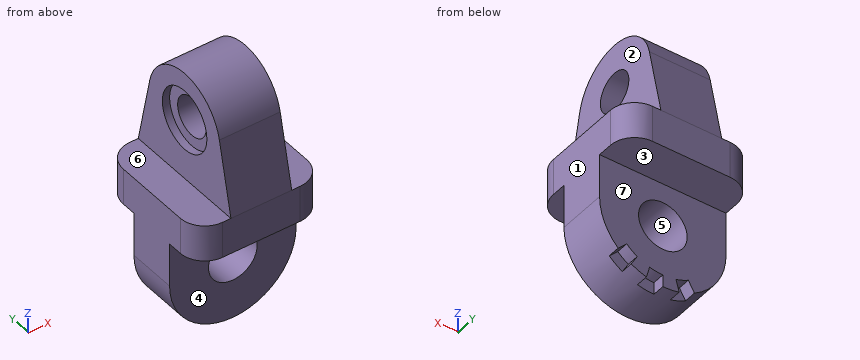
```python
from build123d import *

# Parameters (mm, degrees)
ROUNDED_BASE_BLOCK_DEPTH   = 15
UPPER_BLOCK_DEPTH          = 52
UPPER_BLOCK_NOTCH_A_DEPTH  = 13.5
UPPER_START                = -13.5
UPPER_BLOCK_NOTCH_B_DEPTH  = 13.5
CROSS_BLOCK_DEPTH          = 52
CROSS_BLOCK_NOTCH_A_DEPTH  = 16
CROSS_START                = -16
CROSS_BLOCK_NOTCH_B_DEPTH  = 16
BORE_NOTCH_TEETH_CUT_DEPTH = 5
CROSS_BORE_10_SKETCH_R     = 10
CROSS_BORE_10_DEPTH        = 50
COUNTERBORE_25_SKETCH_R    = 12.5
COUNTERBORE_25_X3_DEPTH    = 3
MAIN_BORE_16_SKETCH_R      = 8
MAIN_BORE_16_DEPTH         = 50


with BuildPart() as part:
    # Base Block Profile Sketch → Rounded Base Block (new body)
    with BuildSketch(Plane.XY):
        with BuildLine():
            Line((-16, 0), (16, 0))
            ThreePointArc((16, 0), (23.071067812, 2.928932188), (26, 10))
            Line((26, 10), (26, 42))
            ThreePointArc((26, 42), (23.071067812, 49.071067812), (16, 52))
            Line((16, 52), (-16, 52))
            ThreePointArc((-16, 52), (-23.071067812, 49.071067812), (-26, 42))
            Line((-26, 42), (-26, 10))
            ThreePointArc((-26, 10), (-23.071067812, 2.928932188), (-16, 0))
        make_face()
    extrude(amount=ROUNDED_BASE_BLOCK_DEPTH)

    # Upper Block Profile Sketch → Upper Block (add)
    with BuildSketch(Plane.ZY.offset(26)):
        with BuildLine():
            Line((15, 52), (15, 0))
            Line((15, 0), (44.311040938, 6.470152944))
            ThreePointArc((44.311040938, 6.470152944), (60, 26), (44.311040938, 45.529847056))
            Line((44.311040938, 45.529847056), (15, 52))
        make_face()
    extrude(amount=-UPPER_BLOCK_DEPTH)

    # Upper Block Notch A Sketch → Upper Block Notch A (cut)
    with BuildSketch(Plane.ZY.offset(26)):
        with BuildLine():
            Line((15, 52), (44.311040938, 45.529847056))
            ThreePointArc((44.311040938, 45.529847056), (60, 26), (44.311040938, 6.470152944))
            Line((44.311040938, 6.470152944), (15, 0))
            Line((15, 0), (15, 52))
        make_face()
    extrude(amount=-UPPER_BLOCK_NOTCH_A_DEPTH, mode=Mode.SUBTRACT)

    # Upper Block Notch B Sketch → Upper Block Notch B (cut)
    with BuildSketch(Plane(origin=(26, 0, 0), x_dir=(0, 0, -1), z_dir=(1, 0, 0)).offset(UPPER_START)):
        with BuildLine():
            Line((-15, 52), (-15, 0))
            Line((-15, 0), (-44.311040938, 6.470152944))
            ThreePointArc((-44.311040938, 6.470152944), (-60, 26), (-44.311040938, 45.529847056))
            Line((-44.311040938, 45.529847056), (-15, 52))
        make_face()
    extrude(amount=UPPER_BLOCK_NOTCH_B_DEPTH, mode=Mode.SUBTRACT)

    # Cross Block Profile Sketch → Cross Block (add)
    with BuildSketch(Plane(origin=(0, 52, 0), x_dir=(1, 0, 0), z_dir=(0, 1, 0))):
        with BuildLine():
            Line((-26, 0), (-26, 18))
            ThreePointArc((-26, 18), (0, 44), (26, 18))
            Line((26, 18), (26, 0))
            Line((26, 0), (-26, 0))
        make_face()
    extrude(amount=-CROSS_BLOCK_DEPTH)

    # Cross Block Notch A Sketch → Cross Block Notch A (cut)
    with BuildSketch(Plane(origin=(0, 52, 0), x_dir=(1, 0, 0), z_dir=(0, 1, 0))):
        with BuildLine():
            Line((-26, 0), (26, 0))
            Line((26, 0), (26, 18))
            ThreePointArc((26, 18), (0, 44), (-26, 18))
            Line((-26, 18), (-26, 0))
        make_face()
    extrude(amount=-CROSS_BLOCK_NOTCH_A_DEPTH, mode=Mode.SUBTRACT)

    # Cross Block Notch B Sketch → Cross Block Notch B (cut)
    with BuildSketch(Plane.XZ.offset(CROSS_START)):
        with BuildLine():
            Line((-26, 0), (26, 0))
            Line((26, 0), (26, -18))
            ThreePointArc((26, -18), (0, -44), (-26, -18))
            Line((-26, -18), (-26, 0))
        make_face()
    extrude(amount=CROSS_BLOCK_NOTCH_B_DEPTH, mode=Mode.SUBTRACT)

    # Bore Notch Teeth Sketch → Bore Notch Teeth Cut (cut)
    with BuildSketch(Plane(origin=(0, 36, 0), x_dir=(1, 0, 0), z_dir=(0, 1, 0))):
        with BuildLine():
            Line((-5.435199947, 38.284442352), (-6.729295173, 43.114071484))
            ThreePointArc((-6.729295173, 43.114071484), (-9.949769241, 42.020867845), (-13, 40.516660498))
            Line((-13, 40.516660498), (-10.5, 36.186533479))
            ThreePointArc((-10.5, 36.186533479), (-8.03635208, 37.401470183), (-5.435199947, 38.284442352))
        make_face()
        with BuildLine():
            Line((0, 44), (0, 39))
            ThreePointArc((0, 39), (2.741050037, 38.820342089), (5.435199947, 38.284442352))
            Line((5.435199947, 38.284442352), (6.729295173, 43.114071484))
            ThreePointArc((6.729295173, 43.114071484), (3.393680998, 43.777566396), (0, 44))
        make_face()
        with BuildLine():
            ThreePointArc((18.384776311, 36.384776311), (15.827797154, 38.627186848), (13, 40.516660498))
            Line((13, 40.516660498), (10.5, 36.186533479))
            ThreePointArc((10.5, 36.186533479), (12.783990009, 34.660420146), (14.849242405, 32.849242405))
            Line((14.849242405, 32.849242405), (18.384776311, 36.384776311))
        make_face()
    extrude(amount=-BORE_NOTCH_TEETH_CUT_DEPTH, mode=Mode.SUBTRACT)

    # Cross Bore Ø10 Sketch → Cross Bore Ø10 (cut)
    with BuildSketch(Plane(origin=(0, 36, 0), x_dir=(1, 0, 0), z_dir=(0, 1, 0))):
        with Locations(Location((0, 18, 0), (0, 0, 180))):
            Circle(CROSS_BORE_10_SKETCH_R)
    extrude(amount=-CROSS_BORE_10_DEPTH, mode=Mode.SUBTRACT)

    # Counterbore Ø25 Sketch → Counterbore Ø25 x3 (cut)
    with BuildSketch(Plane.ZY.offset(12.5)):
        with Locations(Location((40, 26, 0), (0, 0, 270))):
            Circle(COUNTERBORE_25_SKETCH_R)
    extrude(amount=-COUNTERBORE_25_X3_DEPTH, mode=Mode.SUBTRACT)

    # Main Bore Ø16 Sketch → Main Bore Ø16 (cut)
    with BuildSketch(Plane.ZY.offset(9.5)):
        with Locations(Location((40, 26, 0), (0, 0, 270))):
            Circle(MAIN_BORE_16_SKETCH_R)
    extrude(amount=-MAIN_BORE_16_DEPTH, mode=Mode.SUBTRACT)


solid = part.part
```
Can you work these out from the model? Positions are in its coordinate system, mm. Face numbers are marked on the shaded views. A direction names the side the tool comes from. Round coordinates to 2 decimals unless told otherwise and drop trailing zeros. Order: outer loops, then holes, each group sorted by start corner. A loop starts at its lowest first (then second) coordinate and runs counter-clockwise, first axis right, second up.
(1) If we section it at A-A (y = 26): Please give me the cut outline in (x, z), plus the area to 3 significant figures.
Results are:
outline: (-26, -18) arc R26 ccw to (26, -18) - (26, 15) - (12.5, 15) - (12.5, 32) - (-9.5, 32) - (-9.5, 27.5) - (-12.5, 27.5) - (-12.5, 15) - (-26, 15) - close; (-12.5, 52.5) - (-9.5, 52.5) - (-9.5, 48) - (12.5, 48) - (12.5, 60) - (-12.5, 60) - close; hole circle Ø20 at (0, -18)
area: 3,160 mm2
(2) We'd pull the mould along Z, two halves only. Please class the marked faces 5, 6 and 7: +Z half, -Z half, draft (parallel to the pull), parting line (faces both ways), or undercut.
Results are:
face 5: undercut
face 6: +Z half
face 7: draft
(3) If we section it at D-D (x = -22.5): Please give me the cut outline in (y, z).
Results are:
outline: (2.4, 0) - (16, 0) - (16, -31.03) - (36, -31.03) - (36, 0) - (49.6, 0) - (49.6, 15) - (2.4, 15) - close
(4) If we section it at B-B (z = 40): Please give me the cut outline in (x, y).
Results are:
outline: (-12.5, 5.52) - (12.5, 5.52) - (12.5, 18) - (-9.5, 18) - (-9.5, 13.5) - (-12.5, 13.5) - close; (-12.5, 38.5) - (-9.5, 38.5) - (-9.5, 34) - (12.5, 34) - (12.5, 46.48) - (-12.5, 46.48) - close
(5) If we section it at C-C (z = 12): Please give me the cut outline in (x, y), plus the area to 3 significant figures.
Results are:
outline: (-26, 10) arc R10 ccw to (-16, 0) - (16, 0) arc R10 ccw to (26, 10) - (26, 42) arc R10 ccw to (16, 52) - (-16, 52) arc R10 ccw to (-26, 42) - close
area: 2,620 mm2
(6) I'm going to push flat-ended pins straight in: pin 1 (4 mm diameter, centred on y = 34.5, z = -41.5, fed in from +X); pin 2 (10 mm diameter, centred on x = -4.5, y = 36.5, fed in from +Z); pin 3 (8 mm diameter, centred on y = 14, z = 32, fed in from -X); pin 4 (9.5 mm diameter, centred on y = 26, z = 40, fed in from +X). Where does each tip first touch, or does it pass through?
Results are:
pin 1: stops at x = 13
pin 2: stops at z = 59.23
pin 3: stops at x = -12.5
pin 4: passes through
(7) If I drill on L1, parallel to Z at x = -3.75, y = 26; L2, parallel to Y at x = 6, z = -36; L3, parallel to Z at x = 24, y = 32.5, over which ranges is the centre line in solid material (lowest first)?
Results are:
L1: z = -43.73 to -27.27, -8.73 to 32, 48 to 60
L2: y = 16 to 36
L3: z = -28 to 15
(8) On a 3-axis mill with a long thin cutter (end or side, diameter ignored), from which of +Z, -Z, +X, -X, +Y, -Y can I reach the whole of each face in a straight line? I mean the marked faces 1, 2, 3 and 4. Say none if no direction works.
Results are:
face 1: +Z, -Z, +X, +Y, -Y
face 2: +Z, +X, +Y, -Y
face 3: -Z, +X, -X, +Y
face 4: -Z, +X, -X, -Y
